from build123d import *

# Parameters (mm, degrees)
EXTRUDE_1_DEPTH = 12


with BuildPart() as part:
    # 草图1 → 凸台-拉伸1 (new body)
    with BuildSketch(Plane.XY):
        Polygon((0, 9), (0, 0), (1.8, 0), (1.8, 7.7), (0.5, 9), align=None)
    extrude(amount=EXTRUDE_1_DEPTH)


solid = part.part
Work out the finished part from the listing and answer in its coordinate system (mm). Round coordinates to 2 decimals unless told otherwise and drop trailing zeros. Write each loop counter-clockwise with the first axis right and the second up, starting at its lowest first coordinate (ties: lowest second). Pieces come first, ordered by that corner, then holes. Notation, with made-up numbers: (-22, 30) -> (15, 30) arc R35 ccw to (15, 69) -> close; hole circle Ø3 at (12, 24.5). An arc over 180 degrees is marked (long way). Answer as CSV lines item,"result". Start each with the question number.
(1) The part is cut by section B-B, the plane x = 1.2. Give the vertices of the cut face in (y, z).
(2) The part is cut by section A-A, the plane z = 1. Give the vertices of the cut face in (x, y), then the cut area to 3 significant figures.
(3) Find the intervals of material crossed by probe 1 along Y at (x, z) = (0.55, 4.75); probe 2 along Y at (x, z) = (0.85, 2.75); probe 3 along X at (y, z) = (8.25, 6.75), in increasing order.
Output values:
1,outline,"(0, 0) -> (8.3, 0) -> (8.3, 12) -> (0, 12) -> close"
2,outline,"(0, 0) -> (1.8, 0) -> (1.8, 7.7) -> (0.5, 9) -> (0, 9) -> close"
2,area,"15.4 mm²"
3,probe 1,"y = 0 to 8.95"
3,probe 2,"y = 0 to 8.65"
3,probe 3,"x = 0 to 1.25"
